Can you work these out from the model? Positions are in its coordinate system, mm. A direction names the side the tool comes from. Round coordinates to 2 decimals unless told otherwise and drop trailing zeros. Order: outer loops, then holes, each group sorted by start corner. A loop starts at its lowest first (then second) coordinate and runs counter-clockwise, first axis right, second up.
Q1. If I drill on line 1 (Z direction, x = 0, y = -4.4); line 2 (X direction, y = 3, z = 15.5), over which ranges is the centre line in solid material (lowest first)?
Q2. Will these pins go through, and if not, where does the flat tip stop? P1, Ø4.5, axis at x = 0, z = 70, coming from the +Y side; P2, Ø5, axis at x = -1, z = 131.5, coming from the +Y side; P3, Ø9, axis at x = 0, z = 10, coming from the -Y side.
Q3. For faces 4 (the face through (1.122, -4.172, 12.705)), 5 (the face through (0, -1.5, 91)), which set-ups out of +Z, -Z, +X, -X, +Y, -Y let a thin tool reach every point of the face, with its end or its side?
Q4. If we section it at A-A (z = 10): Please give me the cut outline in (x, y), plus the area to 3 significant figures.
Q5. If we section it at B-B (z = 33): Please give me the cut outline in (x, y).
Q6. We'd pull the mould along Z, two halves only. Please class faces 1 (the face through (0, -2, 150)), 2 (the face through (0, -2, 0)), 3 (the face through (-0.88, -4.172, 102.793)): pulls with the +Z half, pulls with the -Z half, needs draft (parallel to the pull), parting line crosses it, or undercut.
from build123d import *

# Parameters (mm, degrees)
BOSS_EXTRUDE1_DEPTH                          = 150
HOLE_SIZE_PER_PHILLIPS_SLOTTED_COUNT_2_COUNT = 2
HOLE_SIZE_PER_PHILLIPS_SLOTTED_COUNT_2_PITCH = 30
LPATTERN1_COUNT                              = 4
LPATTERN1_PITCH                              = 30
CHAMFER1_SIZE                                = 0.3


with BuildPart() as part:
    # Sketch1 → Boss-Extrude1 (new body)
    with BuildSketch(Plane.XY):
        Polygon((-7, 4.5), (-7, -1.5), (7, -1.5), (7, 4.5), (9.5, 4.5), (9.5, -4.5), (-9.5, -4.5), (-9.5, 4.5), align=None)
    extrude(amount=BOSS_EXTRUDE1_DEPTH)

    # Sketch5 → Hole size per Phillips slotted countersunk wood screw type 1 (revolve, cut)
    with BuildSketch(Plane(origin=(0, -1.5, 10), x_dir=(0, 0, 1), z_dir=(1, 0, 0))):
        Polygon((0, 0), (0, 3), (2.75, 3), (2.75, 2.85), (5.6, 0), align=None)
    hole_size_per_phillips_slotted_countersu = revolve(axis=Axis((0, 4.85, 10), (0, -1, 0)), mode=Mode.SUBTRACT)

    # Hole size per Phillips slotted count 2: Hole size per Phillips slotted countersunk wood screw type 1 ×2
    with Locations(*[(0, 0, i * HOLE_SIZE_PER_PHILLIPS_SLOTTED_COUNT_2_PITCH) for i in range(1, HOLE_SIZE_PER_PHILLIPS_SLOTTED_COUNT_2_COUNT)]):
        add(hole_size_per_phillips_slotted_countersu, mode=Mode.SUBTRACT)

    # LPattern1: Hole size per Phillips slotted countersunk wood screw type 1 ×4
    with Locations(*[(0, 0, i * LPATTERN1_PITCH) for i in range(1, LPATTERN1_COUNT)]):
        add(hole_size_per_phillips_slotted_countersu, mode=Mode.SUBTRACT)

    # LPattern1 copy 1 sketch → LPattern1 copy 1 (revolve, cut)
    with BuildSketch(Plane(origin=(0, -1.5, 70), x_dir=(0, 0, 1), z_dir=(1, 0, 0))):
        Polygon((0, 0), (0, 3), (2.75, 3), (2.75, 2.85), (5.6, 0), align=None)
    revolve(axis=Axis((0, 4.85, 70), (0, -1, 0)), mode=Mode.SUBTRACT)

    # LPattern1 copy 2 sketch → LPattern1 copy 2 (revolve, cut)
    with BuildSketch(Plane(origin=(0, -1.5, 100), x_dir=(0, 0, 1), z_dir=(1, 0, 0))):
        Polygon((0, 0), (0, 3), (2.75, 3), (2.75, 2.85), (5.6, 0), align=None)
    revolve(axis=Axis((0, 4.85, 100), (0, -1, 0)), mode=Mode.SUBTRACT)

    # LPattern1 copy 3 sketch → LPattern1 copy 3 (revolve, cut)
    with BuildSketch(Plane(origin=(0, -1.5, 130), x_dir=(0, 0, 1), z_dir=(1, 0, 0))):
        Polygon((0, 0), (0, 3), (2.75, 3), (2.75, 2.85), (5.6, 0), align=None)
    revolve(axis=Axis((0, 4.85, 130), (0, -1, 0)), mode=Mode.SUBTRACT)

    # Chamfer1
    chamfer1_edges = [part.edges().sort_by_distance(p)[0] for p in [
        (9.5, 4.5, 75),
        (-9.5, 4.5, 75),
        (-7, 4.5, 75),
        (7, 4.5, 75),
    ]]
    chamfer(chamfer1_edges, length=CHAMFER1_SIZE)


solid = part.part
Solution:
1. line 1: z = 0 to 7.25, 12.75 to 37.25, 42.75 to 67.25, 72.75 to 97.25, 102.75 to 127.25, 132.75 to 150
1. line 2: x = -9.5 to -7, 7 to 9.5
2. P1: passes through
2. P2: stops at y = -2.8
2. P3: stops at y = -4.5
3. face 4: +Y
3. face 5: +Z, -Z, +Y
4. outline: (-9.5, -4.5) - (-2.75, -4.5) - (-2.75, -4.35) - (-5.6, -1.5) - (-7, -1.5) - (-7, 4.2) - (-7.3, 4.5) - (-9.2, 4.5) - (-9.5, 4.2) - close; (2.75, -4.5) - (9.5, -4.5) - (9.5, 4.2) - (9.2, 4.5) - (7.3, 4.5) - (7, 4.2) - (7, -1.5) - (5.6, -1.5) - (2.75, -4.35) - close
4. area: 62.2 mm2
5. outline: (-9.5, -4.5) - (9.5, -4.5) - (9.5, 4.2) - (9.2, 4.5) - (7.3, 4.5) - (7, 4.2) - (7, -1.5) - (-7, -1.5) - (-7, 4.2) - (-7.3, 4.5) - (-9.2, 4.5) - (-9.5, 4.2) - close
6. face 1: pulls with the +Z half
6. face 2: pulls with the -Z half
6. face 3: undercut
